Geometry: final body of the model. Coordinates: model frame, mm. Give positions to 0.01 mm unless a question says otherwise; leave off trailing zeros. Loops run counter-clockwise (first coordinate to the right, second up) from the corner with the lowest first, then second, coordinate; pieces in that order, holes last. Notation, with made-up numbers: M -36,-1.75 L 4,-1.75 A28 ccw 4,34.25 Z; hole C 1,3 d2. An arc over 180 degrees is marked long. Put each result on its own line as item: value.
```python
from build123d import *

# Parameters (mm, degrees)
SKETCH1_W             = 60
SKETCH1_H             = 50
BOSS_EXTRUDE1_DEPTH   = 14
M8_TAPPED_HOLE1_D     = 6.8
M8_TAPPED_HOLE1_DEPTH = 19.75
M8_TAPPED_HOLE1_TIP   = 2.042926105


with BuildPart() as part:
    # Sketch1 → Boss-Extrude1 (new body)
    with BuildSketch(Plane.XY):
        Rectangle(SKETCH1_W, SKETCH1_H)
    extrude(amount=BOSS_EXTRUDE1_DEPTH)

    # M8 Tapped Hole1
    with Locations(Plane.XY.offset(14)):
        with Locations((-15, 0), (15, 0)):
            Hole(M8_TAPPED_HOLE1_D / 2, depth=M8_TAPPED_HOLE1_DEPTH)
            with Locations((0, 0, -(M8_TAPPED_HOLE1_DEPTH + M8_TAPPED_HOLE1_TIP / 2))):  # 118° drill point
                Cone(0, M8_TAPPED_HOLE1_D / 2, M8_TAPPED_HOLE1_TIP, mode=Mode.SUBTRACT)


solid = part.part
```
Item 1: Line query: probe 1 along X at (y, z) = (2, 11.25); probe 2 along Y at (x, z) = (-15, 10.75); probe 3 along Y at (x, z) = (13, 7.5). Output: solid intervals per line, ascending. Write a range as [from, to].
Output values:
probe 1: [-30, -17.75], [-12.25, 12.25], [17.75, 30]
probe 2: [-25, -3.4], [3.4, 25]
probe 3: [-25, -2.75], [2.75, 25]
Item 2: Section D-D on x = 17. Output: boundary loops of the cut face in (y, z).
Output values:
outline: M -25,0 L -2.75,0 L -2.75,14 L -25,14 Z; M 2.75,0 L 25,0 L 25,14 L 2.75,14 Z
Item 3: Mould query, pull axis Y, two halves, no side actions, for faces 1 (the flat face through (0, 25, 7)), 2 (the flat face through (0, -25, 7)), 3 (the cylindrical face through (17.698, -2.069, 6.902)). Classes: pulls with the +Y half, pulls with the -Y half, needs draft (parallel to the pull), parting line crosses it, or undercut.
Output values:
face 1: pulls with the +Y half
face 2: pulls with the -Y half
face 3: undercut
Item 4: Section A-A on y = 0. Output: boundary loops of the cut face in (x, z).
Output values:
outline: M -30,0 L -18.4,0 L -18.4,14 L -30,14 Z; M -11.6,0 L 11.6,0 L 11.6,14 L -11.6,14 Z; M 18.4,0 L 30,0 L 30,14 L 18.4,14 Z
Item 5: Section C-C on z = 11. Output: boundary loops of the cut face in (x, y).
Output values:
outline: M -30,-25 L 30,-25 L 30,25 L -30,25 Z; hole C -15,0 d6.8; hole C 15,0 d6.8
Item 6: Section B-B on x = -15. Output: boundary loops of the cut face in (y, z).
Output values:
outline: M -25,0 L -3.4,0 L -3.4,14 L -25,14 Z; M 3.4,0 L 25,0 L 25,14 L 3.4,14 Z
